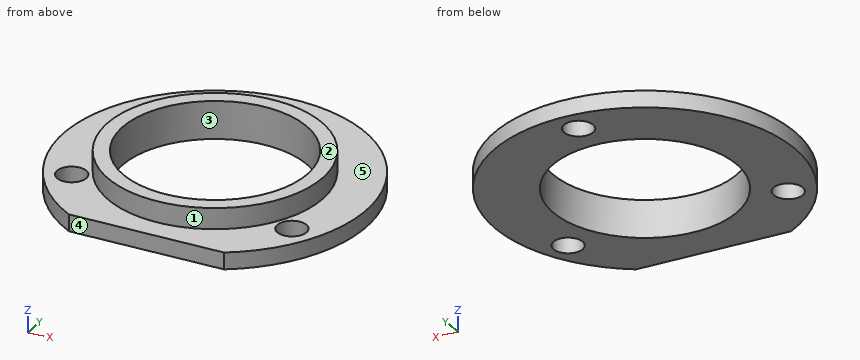
```python
from build123d import *

# Parameters (mm, degrees)
SKETCH_1_R          = 18
SKETCH_1_R_2        = 11
EXTRUDE_1_DEPTH     = 4.5
SKETCH_2_OUTSIDE_W  = 48.222
SKETCH_2_OUTSIDE_H  = 48.222
SKETCH_2_OUTSIDE_R  = 12.8
CUT_EXTRUDE_1_DEPTH = 2.5
SKETCH_3_W          = 45.784626658
SKETCH_3_H          = 5.372844692
CUT_EXTRUDE_2_DEPTH = 26.578311125
SKETCH_4_R          = 1.75
CUT_EXTRUDE_3_DEPTH = 26.850531909


with BuildPart() as part:
    # 草图1 → 凸台-拉伸1 (new body)
    with BuildSketch(Plane.XY):
        Circle(SKETCH_1_R)
        Circle(SKETCH_1_R_2, mode=Mode.SUBTRACT)
    extrude(amount=EXTRUDE_1_DEPTH)

    # 草图2 outside → 切除-拉伸1 (cut)
    with BuildSketch(Plane.XY.offset(4.5)):
        Rectangle(SKETCH_2_OUTSIDE_W, SKETCH_2_OUTSIDE_H)
        Circle(SKETCH_2_OUTSIDE_R, mode=Mode.SUBTRACT)
    extrude(amount=-CUT_EXTRUDE_1_DEPTH, mode=Mode.SUBTRACT)

    # 草图3 → 切除-拉伸2 (cut, through all)
    with BuildSketch(Plane.XY.offset(2)):
        with Locations((-1.895541868, -18.186422346)):
            Rectangle(SKETCH_3_W, SKETCH_3_H)
    extrude(amount=-CUT_EXTRUDE_2_DEPTH, mode=Mode.SUBTRACT)

    # 草图4 → 切除-拉伸3 (cut, through all)
    with BuildSketch(Plane(origin=(0, 0, 0), x_dir=(-1, 0, 0), z_dir=(0, 0, -1))):
        with Locations((0, 15)):
            Circle(SKETCH_4_R)
        with Locations((-12.990381057, -7.5)):
            Circle(SKETCH_4_R)
        with Locations((12.990381057, -7.5)):
            Circle(SKETCH_4_R)
    extrude(amount=-CUT_EXTRUDE_3_DEPTH, mode=Mode.SUBTRACT)


solid = part.part
```
Model file for the job. Use its own axes, mm. Face numbers are marked on the shaded views. A direction names the side the tool comes from. Coordinates: 2 decimals unless noted, no trailing zeros. Write each loop counter-clockwise with the first axis right and the second up, starting at its lowest first coordinate (ties: lowest second). Pieces come first, ordered by that corner, then holes. Notation, with made-up numbers: (84, 79.25) - (113, 79.25) arc R23 cw to (113, 118.25) - close; hole circle Ø4 at (48.5, 46.25). An arc over 180 degrees is marked (long way). Use a Markdown table: item, result. Add a question column.
Item 1: Band-saw the part on B-B, the plane x = 0. Write the cut outline in (y, z), and give its area (3 significant figures).
Item 2: Band-saw the part on C-C, the plane x = 8. Write the cut outline in (y, z).
Item 3: Band-saw the part on D-D, the plane z = 3.9. Write the cut outline in (x, y), and give its area (3 significant figures).
Item 4: 3-axis set-ups, long thin cutter, end or side, ignore diameter. For the marked faces 4 and 5: which of +Z, -Z, +X, -X, +Y, -Y reach the whole face in a straight line?
Item 5: Drop flat-ended pins along their axis: pin 1 (13 mm diameter, centred on x = 0, y = 0, fed in from -Z); pin 2 (6 mm diameter, centred on x = -12.5, y = -8.5, fed in from -Z). Give the stop position or say it passes through.
Item 6: Two-plate mould, pull along Y, no slides. Class the marked faces 1, 2 and 3: pulls with the +Y half, pulls with the -Y half, needs draft (parallel to the pull), parting line crosses it, or undercut.
Item 7: Band-saw the part on A-A, the plane y = 0. Write the cut outline in (x, z).
Item 8: Drill centre lines: line 1 along Y through (x, z) = (0, 1); line 2 along X through (y, z) = (-9, 0.45); line 3 along Y through (x, z) = (0, 3.8). Where is each one in solid material? Low to high.
A:
| question | item | result |
|---|---|---|
| 1 | outline | (-15.5, 0) - (-11, 0) - (-11, 4.5) - (-12.8, 4.5) - (-12.8, 2) - (-15.5, 2) - close; (11, 0) - (13.25, 0) - (13.25, 2) - (12.8, 2) - (12.8, 4.5) - (11, 4.5) - close; (16.75, 0) - (18, 0) - (18, 2) - (16.75, 2) - close |
| 1 | area | 25.0 mm² |
| 2 | outline | (-15.5, 0) - (-7.55, 0) - (-7.55, 4.5) - (-9.99, 4.5) - (-9.99, 2) - (-15.5, 2) - close; (7.55, 0) - (16.12, 0) - (16.12, 2) - (9.99, 2) - (9.99, 4.5) - (7.55, 4.5) - close |
| 3 | outline | circle Ø25.6 at (0, 0); hole circle Ø22 at (0, 0) |
| 3 | area | 135 mm² |
| 4 | face 4 | +Z, -Z, +X, -X, -Y |
| 4 | face 5 | +Z |
| 5 | pin 1 | passes through |
| 5 | pin 2 | stops at z = 0 |
| 6 | face 1 | parting line crosses it |
| 6 | face 2 | needs draft |
| 6 | face 3 | undercut |
| 7 | outline | (-18, 0) - (-11, 0) - (-11, 4.5) - (-12.8, 4.5) - (-12.8, 2) - (-18, 2) - close; (11, 0) - (18, 0) - (18, 2) - (12.8, 2) - (12.8, 4.5) - (11, 4.5) - close |
| 8 | line 1 | y = -15.5 to -11, 11 to 13.25, 16.75 to 18 |
| 8 | line 2 | x = -15.59 to -13.89, -12.09 to -6.32, 6.32 to 12.09, 13.89 to 15.59 |
| 8 | line 3 | y = -12.8 to -11, 11 to 12.8 |
